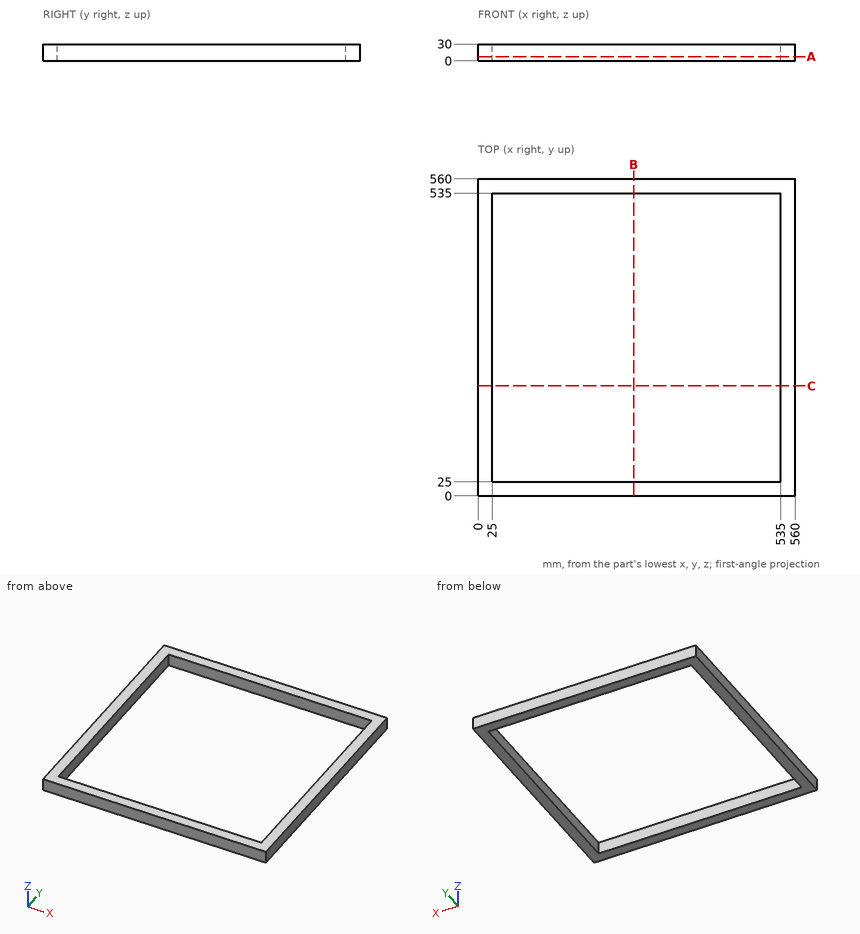
Answer from the drawing. Dimensions are ordinates in mm from the lowest x, y and z of the part. Give positions to 0.01 mm unless a question says otherwise; leave off trailing zeros. Loops run counter-clockwise (first coordinate to the right, second up) from the corner with the lowest first, then second, coordinate; pieces in that order, holes last. Notation, with made-up numbers: (-12, 19.25) -> (-8, 19.25) arc R17 ccw to (-8, 46.25) -> close; hole circle Ø10 at (85, 44). An arc over 180 degrees is marked (long way). Use a Markdown table: item, result.
Q1. Find the intervals of material crossed by line 1 along Y through (x, z) = (534.5, 10), in increasing order.
Solved:
| item | result |
|---|---|
| line 1 | y = 0 to 25, 535 to 560 |
Q2. Section B-B, the plane x = 275 is taken. Determine the outline of the cut face in (y, z), then the cut area to 3 significant figures.
Solved:
| item | result |
|---|---|
| outline | (0, 0) -> (25, 0) -> (25, 30) -> (0, 30) -> close; (535, 0) -> (560, 0) -> (560, 30) -> (535, 30) -> close |
| area | 1,500 mm^2 |
Q3. Section A-A, the plane z = 7.75 is taken. Determine the outline of the cut face in (x, y).
Solved:
| item | result |
|---|---|
| outline | (0, 0) -> (560, 0) -> (560, 560) -> (0, 560) -> close; hole (25, 25) -> (535, 25) -> (535, 535) -> (25, 535) -> close |
